```python
from build123d import *

# Parameters (mm, degrees)
EXTRUDE_1_DEPTH     = 58
SKETCH_2_R          = 2.2
CUT_EXTRUDE_1_DEPTH = 10


with BuildPart() as part:
    # 草图1 → 凸台-拉伸1 (new body)
    with BuildSketch(Plane.XY):
        with BuildLine():
            Line((-3.011664558, 4.541522048), (1.988335442, 4.541522048))
            Line((1.988335442, 4.541522048), (1.988335442, -7.975163179))
            ThreePointArc((1.988335442, -7.975163179), (-1.018873776, -9.651157386), (-3.011664558, -12.458477952))
            Line((-3.011664558, -12.458477952), (-3.011664558, 4.541522048))
        make_face()
    extrude(amount=EXTRUDE_1_DEPTH)

    # 草图2 → 切除-拉伸1 (cut)
    with BuildSketch(Plane(origin=(1.988335442, 0, 0), x_dir=(0, 0, -1), z_dir=(1, 0, 0))):
        with Locations(Location((-19, -0.458477952, 0), (0, 0, 90))):
            Circle(SKETCH_2_R)
        with Locations(Location((-39, -0.458477952, 0), (0, 0, 90))):
            Circle(SKETCH_2_R)
    extrude(amount=-CUT_EXTRUDE_1_DEPTH, mode=Mode.SUBTRACT)


solid = part.part
```
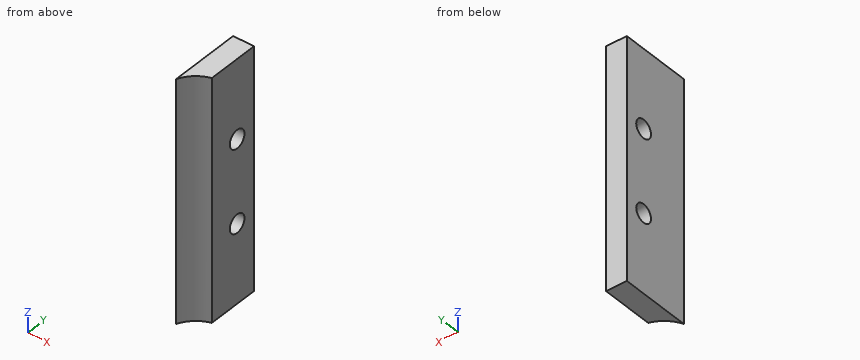
For this review, take the finished solid that the model builds, in its own axes (mm). Coordinates: 2 decimals unless noted, no trailing zeros. Write each loop counter-clockwise with the first axis right and the second up, starting at its lowest first coordinate (ties: lowest second). Pieces come first, ordered by that corner, then holes. Notation, with made-up numbers: (88, 28.25) -> (109, 28.25) arc R18 ccw to (109, 61.25) -> close; hole circle Ø1 at (53, -29.5). An arc over 180 degrees is marked (long way). Put each result on its own line as item: value.
Q1. Take a section at C-C, the plane x = 0.95. State the section outline as (y, z) points, then the cut area to 3 significant figures.
From the geometry:
outline: (-8.36, 0) -> (4.54, 0) -> (4.54, 58) -> (-8.36, 58) -> close; hole circle Ø4.4 at (-0.46, 19); hole circle Ø4.4 at (-0.46, 39)
area: 718 mm2
Q2. Wall thickness on L1, parallel to Z at x = -1.95, y = -2.25; L2, parallel to Z at x = 1.5, y = 0; L3, parallel to Y at x = 1.75, z = 19.5: over which ranges is each line inside the solid? List them lowest first.
From the geometry:
L1: z = 0 to 17.72, 20.28 to 37.72, 40.28 to 58
L2: z = 0 to 16.85, 21.15 to 36.85, 41.15 to 58
L3: y = -8.05 to -2.6, 1.68 to 4.54
Q3. Take a section at B-B, the plane y = -0.25. State the section outline as (x, z) points.
From the geometry:
outline: (-3.01, 0) -> (1.99, 0) -> (1.99, 16.81) -> (-3.01, 16.81) -> close; (-3.01, 21.19) -> (1.99, 21.19) -> (1.99, 36.81) -> (-3.01, 36.81) -> close; (-3.01, 41.19) -> (1.99, 41.19) -> (1.99, 58) -> (-3.01, 58) -> close
Q4. Take a section at D-D, the plane z = 31. State the section outline as (x, y) points.
From the geometry:
outline: (-3.01, -12.46) arc R7.8 cw to (1.99, -7.98) -> (1.99, 4.54) -> (-3.01, 4.54) -> close
Q5. Take a section at A-A, the plane z = 39. State the section outline as (x, y) points, then the cut area to 3 significant figures.
From the geometry:
outline: (-3.01, -12.46) arc R7.8 cw to (1.99, -7.98) -> (1.99, -2.66) -> (-3.01, -2.66) -> close; (-3.01, 1.74) -> (1.99, 1.74) -> (1.99, 4.54) -> (-3.01, 4.54) -> close
area: 48.4 mm2
Q6. Clearance check with flat-ended pins moving along their axes: pin 1 Ø2.5 at (y, z) = (-0.46, 39) entering from -X; pin 2 Ø3 at (x, y) = (-1, -10.5) entering from +Z; pin 3 Ø2 at (x, z) = (-1.5, 17.5) entering from -Y. State where each tip first meets the part, or that it passes through.
From the geometry:
pin 1: passes through
pin 2: stops at z = 58
pin 3: stops at y = -11.45
